Can you work these out from the drawing? Everything is in mm from the part's minimum corner. Round coordinates to 2 decimals unless told otherwise and drop trailing zeros. Loops run counter-clockwise (first coordinate to the right, second up) from the corner with the lowest first, then second, coordinate; pieces in that order, holes last. Notation, with made-up numbers: (-21, -26.75) -> (-9, -26.75) arc R5 cw to (-9, -21.75) -> close; hole circle Ø5 at (5, 32). An arc over 180 degrees is marked (long way). One line per item, written item: value.
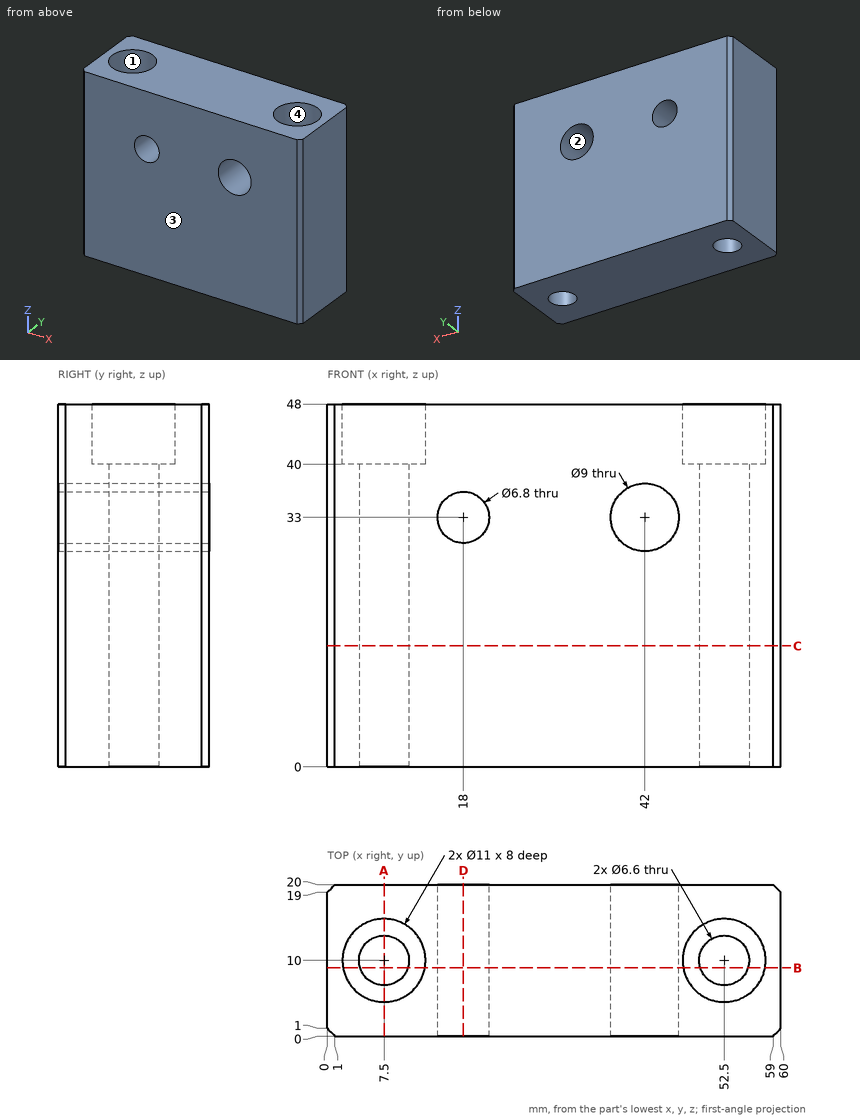
Item 1: If we section it at A-A on x = 7.5: List the corners of the cut face in (y, z) for me, plus the area to 3 significant figures.
Output:
outline: (0, 0) -> (6.7, 0) -> (6.7, 40) -> (4.5, 40) -> (4.5, 48) -> (0, 48) -> close; (13.3, 0) -> (20, 0) -> (20, 48) -> (15.5, 48) -> (15.5, 40) -> (13.3, 40) -> close
area: 608 mm²
Item 2: If we section it at C-C on z = 16: List the corners of the cut face in (x, y) for me.
Output:
outline: (0, 1) -> (1, 0) -> (59, 0) -> (60, 1) -> (60, 19) -> (59, 20) -> (1, 20) -> (0, 19) -> close; hole circle Ø6.6 at (7.5, 10); hole circle Ø6.6 at (52.5, 10)
Item 3: If we section it at B-B on y = 9: List the corners of the cut face in (x, z) for me.
Output:
outline: (0, 0) -> (4.36, 0) -> (4.36, 40) -> (2.09, 40) -> (2.09, 48) -> (0, 48) -> close; (10.64, 0) -> (49.36, 0) -> (49.36, 40) -> (47.09, 40) -> (47.09, 48) -> (12.91, 48) -> (12.91, 40) -> (10.64, 40) -> close; (55.64, 0) -> (60, 0) -> (60, 48) -> (57.91, 48) -> (57.91, 40) -> (55.64, 40) -> close; hole circle Ø6.8 at (18, 33); hole circle Ø9 at (42, 33)
Item 4: If we section it at D-D on x = 18: List the corners of the cut face in (y, z) for me.
Output:
outline: (0, 0) -> (20, 0) -> (20, 29.6) -> (0, 29.6) -> close; (0, 36.4) -> (20, 36.4) -> (20, 48) -> (0, 48) -> close
Item 5: Will this pin go through, and if not, where does the flat tip stop? pin 1 Ø9 at (x, y) = (52.5, 10) entering from +Z.
Output:
pin 1: stops at z = 40
Item 6: If we mould it in two halves opening along Y, with no side actions, what happens to the marked faces 1, 2, 3 and 4? For each: released by +Y, released by -Y, zero draft, split by the parting line, or undercut.
Output:
face 1: undercut
face 2: zero draft
face 3: released by -Y
face 4: undercut
Item 7: I need wall thicknesses on line 1 (Z direction, x = 18, y = 5); line 2 (X direction, y = 13.5, z = 32.5); line 3 (Z direction, x = 42, y = 4.25). Which ranges of each line are inside material? Lowest first, please. Write a range as from..to.
Output:
line 1: z = 0..29.6, 36.4..48
line 2: x = 0..14.64, 21.36..37.53, 46.47..60
line 3: z = 0..28.5, 37.5..48
